from build123d import *

# Parameters (mm, degrees)
SKETCH_2_W                   = 75
SKETCH_2_H                   = 32
EXTRUDE_1_DEPTH              = 70
SKETCH_4_R                   = 26.05
CUT_EXTRUDE_1_DEPTH          = 82.007715682
HOLE_WIZARD_M5_1_D           = 5.5
HOLE_WIZARD_M5_1_CBORE_D     = 10
HOLE_WIZARD_M5_1_CBORE_DEPTH = 27
SKETCH_7_W                   = 17
SKETCH_7_H                   = 20
CUT_EXTRUDE_2_DEPTH          = 104.831594421
HOLE_WIZARD_M5_1_2_D         = 4.2
HOLE_WIZARD_M5_1_2_DEPTH     = 12.4
HOLE_WIZARD_M5_1_2_TIP       = 1.2618073


with BuildPart() as part:
    # 草图2 → 凸台-拉伸1 (new body)
    with BuildSketch(Plane.XY):
        Rectangle(SKETCH_2_W, SKETCH_2_H)
    extrude(amount=EXTRUDE_1_DEPTH)

    # 草图4 → 切除-拉伸1 (cut, through all)
    with BuildSketch(Plane.XY.offset(70)):
        with Locations((0, 16)):
            Circle(SKETCH_4_R)
    extrude(amount=-CUT_EXTRUDE_1_DEPTH, mode=Mode.SUBTRACT)

    # Hole Wizard M5 _1 (through all)
    with Locations(Plane(origin=(0, 16, 0), x_dir=(1, 0, 0), z_dir=(0, 1, 0))):
        with Locations((-31.775, -8), (-31.775, -62), (31.775, -62), (31.775, -8)):
            CounterBoreHole(HOLE_WIZARD_M5_1_D / 2, HOLE_WIZARD_M5_1_CBORE_D / 2, HOLE_WIZARD_M5_1_CBORE_DEPTH)

    # 草图7 → 切除-拉伸2 (cut, through all)
    with BuildSketch(Plane.ZY.offset(37.5)):
        with Locations((61.5, 6)):
            Rectangle(SKETCH_7_W, SKETCH_7_H)
    extrude(amount=-CUT_EXTRUDE_2_DEPTH, mode=Mode.SUBTRACT)

    # Hole Wizard M5 _1 2
    with Locations(Plane(origin=(0, 16, 0), x_dir=(1, 0, 0), z_dir=(0, 1, 0))):
        with Locations((-31.75, -21), (-31.75, -45), (31.75, -21), (31.75, -45)):
            Hole(HOLE_WIZARD_M5_1_2_D / 2, depth=HOLE_WIZARD_M5_1_2_DEPTH)
            with Locations((0, 0, -(HOLE_WIZARD_M5_1_2_DEPTH + HOLE_WIZARD_M5_1_2_TIP / 2))):  # 118° drill point
                Cone(0, HOLE_WIZARD_M5_1_2_D / 2, HOLE_WIZARD_M5_1_2_TIP, mode=Mode.SUBTRACT)


solid = part.part
For this review, take the finished solid that the model builds, in its own axes (mm). A direction names the side the tool comes from. Coordinates: 2 decimals unless noted, no trailing zeros. Loops run counter-clockwise (first coordinate to the right, second up) from the corner with the lowest first, then second, coordinate; pieces in that order, holes last. Notation, with made-up numbers: (38.25, 31) - (44.25, 31) arc R23 ccw to (44.25, 64) - close; hole circle Ø7 at (24.5, 26). An arc over 180 degrees is marked (long way). Return JSON: item names as keys, results as strings.
Item 1: Mouldability with a two-part tool opening along Z and no side actions: class faces 1 (the flat face through (-30, 4, 53)), 2 (the flat face through (-0.5, -10.4, 0)), 3 (the cylindrical face through (28.09, 2.69, 4.62)), 4 (the flat face through (32, 16, 26)) as pulls with the +Z half, pulls with the -Z half, needs draft (parallel to the pull), parting line crosses it, or undercut.
Determined:
{"face 1": "pulls with the +Z half", "face 2": "pulls with the -Z half", "face 3": "undercut", "face 4": "needs draft"}
Item 2: For line 1 (Z direction, x = -31.75, y = 8.25); line 2 (Z direction, x = 31.5, y = -7.5); line 3 (Z direction, x = -30, y = -10.5), list the stretches that pass through material, from the lowest coordinate up.
Determined:
{"line 1": "z = 0 to 3, 13 to 18.9, 23.1 to 42.9, 47.1 to 53", "line 2": "z = 0 to 3.01, 12.99 to 57.01, 66.99 to 70", "line 3": "z = 0 to 3.33, 12.67 to 57.33, 66.67 to 70"}
Item 3: Take a section at B-B (y = -12.5). Give the boundary of the cut face in (x, z) (3 decimals).
Determined:
{"outline": "(-37.5, 0) - (37.5, 0) - (37.5, 70) - (-37.5, 70) - close; hole circle Ø5.5 at (-31.775, 8); hole circle Ø5.5 at (-31.775, 62); hole circle Ø5.5 at (31.775, 8); hole circle Ø5.5 at (31.775, 62)"}
Item 4: Insertion check: pin 1 (4 mm diameter, centred on x = 31.75, z = 45, fed in from +Y); pin 2 (6 mm diameter, centred on x = -27, y = 4.5, fed in from +Z); pin 3 (12 mm diameter, centred on x = -11.5, z = 13, fed in from +Y); pin 4 (5 mm diameter, centred on x = -31.775, z = 62, fed in from -Y). Each pin has a flat end and moves straight along its axis. Give the tip position at first contact, or say it passes through.
Determined:
{"pin 1": "stops at y = 3.54", "pin 2": "stops at z = 53", "pin 3": "stops at y = -3.3", "pin 4": "passes through"}
Item 5: Take a section at D-D (y = -2.5). Give the boundary of the cut face in (x, z) (3 decimals).
Determined:
{"outline": "(-37.5, 0) - (-18.34, 0) - (-18.34, 53) - (-37.5, 53) - close; (18.34, 0) - (37.5, 0) - (37.5, 53) - (18.34, 53) - close; hole circle Ø10 at (-31.775, 8); hole circle Ø10 at (31.775, 8)"}
Item 6: Take a section at C-C (z = 8). Give the boundary of the cut face in (x, y) (3 decimals), then the cut area to 3 significant figures.
Determined:
{"outline": "(-37.5, -16) - (-34.525, -16) - (-34.525, -11) - (-36.775, -11) - (-36.775, 16) - (-37.5, 16) - close; (-29.025, -16) - (29.025, -16) - (29.025, -11) - (26.775, -11) - (26.775, 16) - (26.05, 16) arc R26.05 cw to (-26.05, 16) - (-26.775, 16) - (-26.775, -11) - (-29.025, -11) - close; (34.525, -16) - (37.5, -16) - (37.5, 16) - (36.775, 16) - (36.775, -11) - (34.525, -11) - close", "area": "739 mm2"}
Item 7: Take a section at A-A (y = 6.5). Give the boundary of the cut face in (x, z) (3 decimals), then the cut area to 3 significant figures.
Determined:
{"outline": "(-37.5, 0) - (-24.256, 0) - (-24.256, 53) - (-37.5, 53) - close; (24.256, 0) - (37.5, 0) - (37.5, 53) - (24.256, 53) - close; hole circle Ø10 at (-31.775, 8); hole circle Ø4.2 at (-31.75, 21); hole circle Ø4.2 at (-31.75, 45); hole circle Ø10 at (31.775, 8); hole circle Ø4.2 at (31.75, 21); hole circle Ø4.2 at (31.75, 45)", "area": "1,190 mm2"}
Item 8: For faces 5 (the flat face through (37.5, 0, 27)), 6 (the cylindrical face through (31.124, -7.451, 57.043)), list the 3-axis set-ups (+Z, -Z, +X, -X, +Y, -Y) from which the entire face can be reached by the end or side of a thin tool; tool diameter is ignored.
Determined:
{"face 5": "+Z, -Z, +X, +Y, -Y", "face 6": "+Y"}
